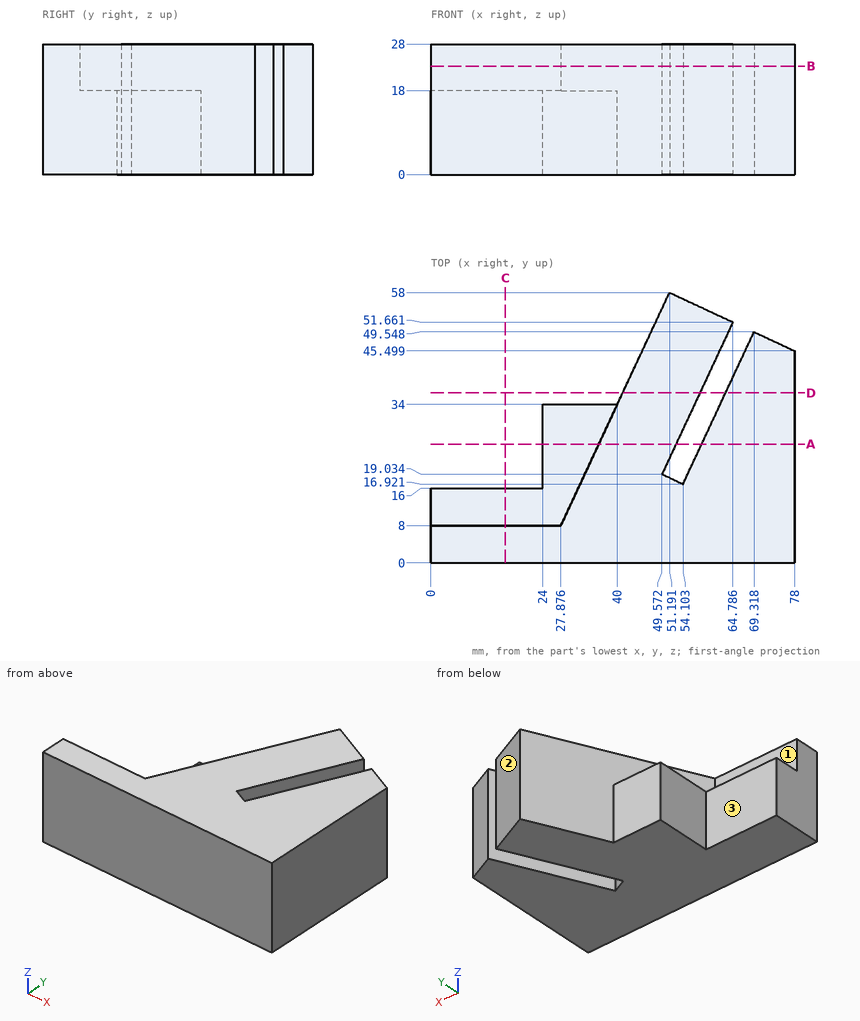
Check sheet for the drawn part. Datum: minimum x, y, z corner. Units: mm. A direction names the side the tool comes from. Round coordinates to 2 decimals unless told otherwise and drop trailing zeros. Write each loop counter-clockwise with the first axis right and the second up, starting at its lowest first coordinate (ties: lowest second). Pieces come first, ordered by that corner, then holes. Notation, with made-up numbers: (34.5, 59) -> (59.5, 59) arc R18 cw to (59.5, 76) -> close; hole circle Ø1 at (31.5, -11.5). An arc over 180 degrees is marked (long way). Write each question's results on one line, items separated by ' | '. Start each with the question number.
1. Cross-section at D-D (y = 36.5). Enter the section's corners in (x, z) (1 decimal).
2. Cross-section at A-A (y = 25.5). Enter the section's corners in (x, z).
3. Cross-section at C-C (x = 16). Enter the section's corners in (y, z), then the cut area to 3 significant figures.
4. Cross-section at B-B (z = 23.25). Enter the section's corners in (x, y).
5. Depth check by flat-ended pin: P1, Ø1.5, axis at y = 45, z = 3, coming from the -X side; P2, Ø4, axis at y = 38.5, z = 19.5, coming from the -X side (1 decimal); P3, Ø11, axis at x = 20.5, z = 21.5, coming from the +Y side. Enter the tip coordinate at first touch or a pass-through.
6. Material ranges on probe 1 along Y at (x, z) = (50.5, 26.75) (1 decimal); probe 2 along X at (y, z) = (31, 1.25); probe 3 along Y at (x, z) = (33, 6.25), recorded low to high. Write a range as from..to.
7. Set-up check for the marked faces 1, 2 and 3: record each of +Z, -Z, +X, -X, +Y, -Y from which the full face is reachable in a straight line by a thin tool's end or side.
Solutions:
1) outline: (41.2, 0) -> (57.7, 0) -> (57.7, 28) -> (41.2, 28) -> close; (63.2, 0) -> (78, 0) -> (78, 28) -> (63.2, 28) -> close
2) outline: (24, 0) -> (52.59, 0) -> (52.59, 28) -> (36.04, 28) -> (36.04, 18) -> (24, 18) -> close; (58.1, 0) -> (78, 0) -> (78, 28) -> (58.1, 28) -> close
3) outline: (0, 0) -> (16, 0) -> (16, 18) -> (8, 18) -> (8, 28) -> (0, 28) -> close | area: 368 mm2
4) outline: (0, 0) -> (78, 0) -> (78, 45.5) -> (69.32, 49.55) -> (54.1, 16.92) -> (49.57, 19.03) -> (64.79, 51.66) -> (51.19, 58) -> (27.88, 8) -> (0, 8) -> close
5) P1: stops at x = 44.78 | P2: stops at x = 41.2 | P3: stops at y = 34
6) probe 1: y = 0..18.6, 21..56.5 | probe 2: x = 24..55.15, 60.67..78 | probe 3: y = 0..34
7) face 1: +Z, -X, +Y | face 2: +Z, -Z, +X, +Y | face 3: +Z, -Z, -X, +Y
